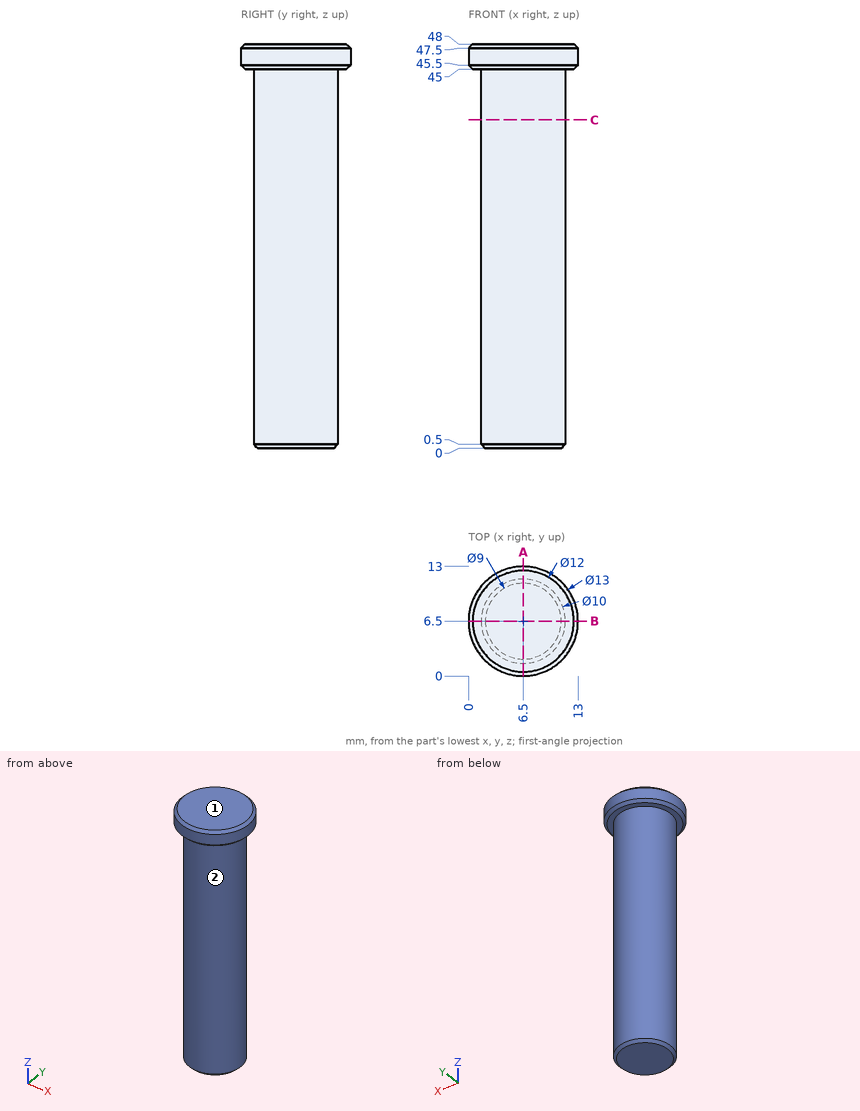
Could you check a few things on this drawing? It's one solid part, dimensions in mm from its lowest x, y, z. A direction names the side the tool comes from. Coordinates: 2 decimals unless noted, no trailing zeros. Order: outer loops, then holes, each group sorted by start corner. A loop starts at its lowest first (then second) coordinate and runs counter-clockwise, first axis right, second up. Notation, with made-up numbers: (42.25, 60.5) -> (96.25, 60.5) arc R35 ccw to (96.25, 92.5) -> close; hole circle Ø2 at (19.25, 59). An arc over 180 degrees is marked (long way). Answer in a Markdown table with one row per item.
(1) On a 3-axis mill with a long thin cutter (end or side, diameter ignored), from which of +Z, -Z, +X, -X, +Y, -Y can I reach the whole of each face in a straight line? I mean the marked faces 1 and 2. Say none if no direction works.
Answer key:
| item | result |
|---|---|
| face 1 | +Z, +X, -X, +Y, -Y |
| face 2 | -Z |
(2) Please list where these lines run through material, in increasing order: probe 1 along Z at (x, y) = (1.75, 3); probe 2 along X at (y, z) = (9.5, 17.5); probe 3 along X at (y, z) = (10.25, 42).
Answer key:
| item | result |
|---|---|
| probe 1 | 45 to 48 |
| probe 2 | 2.5 to 10.5 |
| probe 3 | 3.19 to 9.81 |
(3) I want a section at C-C on z = 39. List the corners of the cut face in (x, y) for me.
Answer key:
| item | result |
|---|---|
| outline | circle Ø10 at (6.5, 6.5) |
(4) I want a section at A-A on x = 6.5. List the corners of the cut face in (y, z) for me.
Answer key:
| item | result |
|---|---|
| outline | (0, 45.5) -> (0.5, 45) -> (1.5, 45) -> (1.5, 0.5) -> (2, 0) -> (11, 0) -> (11.5, 0.5) -> (11.5, 45) -> (12.5, 45) -> (13, 45.5) -> (13, 47.5) -> (12.5, 48) -> (0.5, 48) -> (0, 47.5) -> close |
(5) Will these pins go through, and if not, where does the flat tip stop? pin 1 Ø1 at (y, z) = (10.5, 34.5) entering from +X; pin 2 Ø1 at (y, z) = (4.5, 15) entering from -X; pin 3 Ø5 at (y, z) = (4, 5) entering from +X.
Answer key:
| item | result |
|---|---|
| pin 1 | x = 10.07 |
| pin 2 | x = 1.73 |
| pin 3 | x = 11.5 |
